The model under review builds one solid part; all positions refer to its coordinate system, in mm. A direction names the side the tool comes from. Coordinates: 2 decimals unless noted, no trailing zeros. Order: outer loops, then holes, each group sorted by start corner. A loop starts at its lowest first (then second) coordinate and runs counter-clockwise, first axis right, second up. Notation, with made-up numbers: (-33, 52) -> (-26, 52) arc R24 cw to (-26, 91) -> close; hole circle Ø3 at (81.5, 43). An arc over 180 degrees is marked (long way). Use one line per item in the form item = value. Start each with the question number.
(1) Mouldability with a two-part tool opening along Y and no side actions: class faces 1 (the flat face through (74, 58, -64)), 2 (the flat face through (74, 36, -64)), 3 (the flat face through (64, 32, -83)), 4 (the cylindrical face through (-84, 18, -15)) as +Y half, -Y half, draft (parallel to the pull), parting line (faces both ways), or undercut.
(2) Take a section at B-B (z = -129.5). State the section outline as (x, y) points.
(3) Insertion check: pin 1 Ø13 at (x, z) = (-77.5, -72) entering from +Y; pin 2 Ø2 at (y, z) = (35.5, -105) entering from -X; pin 3 Ø7 at (x, z) = (80, -15) entering from -Y; pin 4 Ø1 at (y, z) = (48.5, -93) entering from -X. Each pin has a flat end and moves straight along its axis. Give the tip position at first contact, or say it passes through.
(4) Take a section at A-A (x = -80). State the section outline as (y, z) points.
(5) Take a section at D-D (x = 0). State the section outline as (y, z) points.
(6) Take a section at C-C (y = 54). State the section outline as (x, z) points, then the cut area to 3 significant figures.
(7) Wall thickness on line 1 along Y through (x, z) = (64.5, -159.5); line 2 along X through (y, z) = (59.5, -161); line 3 along Z through (x, y) = (21, 47.5): over which ranges is each line inside the solid? List them lowest first.
(8) For faces 5 (the flat face through (64, 3, -83)), 6 (the flat face through (90, 47, -35)), 7 (the flat face through (-74, 7, -64)), list the 3-axis set-ups (+Z, -Z, +X, -X, +Y, -Y) from which the entire face can be reached by the end or side of a thin tool; tool diameter is ignored.
```python
from build123d import *

# Parameters (mm, degrees)
BOSS_EXTRUDE1_DEPTH = 65
SKETCH2_R           = 35
CUT_EXTRUDE1_DEPTH  = 65
SKETCH3_W           = 26
SKETCH3_H           = 7
CUT_EXTRUDE2_DEPTH  = 212.482859826
SKETCH4_R           = 4
CUT_EXTRUDE3_DEPTH  = 210.437341465
SKETCH5_W           = 26
SKETCH5_H           = 7
CUT_EXTRUDE4_DEPTH  = 212.482859826


with BuildPart() as part:
    # Sketch1 → Boss-Extrude1 (new body)
    with BuildSketch(Plane(origin=(0, 0, 0), x_dir=(1, 0, 0), z_dir=(0, 1, 0))):
        with BuildLine():
            Line((-90, 0), (90, 0))
            Line((90, 0), (90, 70))
            Line((90, 70), (69.444464042, 156.905307326))
            ThreePointArc((69.444464042, 156.905307326), (58.862371963, 173.528272565), (40.25, 180))
            Line((40.25, 180), (-40.25, 180))
            ThreePointArc((-40.25, 180), (-58.862371963, 173.528272565), (-69.444464042, 156.905307326))
            Line((-69.444464042, 156.905307326), (-90, 70))
            Line((-90, 70), (-90, 0))
        make_face()
    extrude(amount=BOSS_EXTRUDE1_DEPTH)

    # Sketch2 → Cut-Extrude1 (cut)
    with BuildSketch(Plane(origin=(0, 65, 0), x_dir=(1, 0, 0), z_dir=(0, 1, 0))):
        with Locations(Location((0, 117, 0), (0, 0, 270))):
            Circle(SKETCH2_R)
    extrude(amount=-CUT_EXTRUDE1_DEPTH, mode=Mode.SUBTRACT)

    # Sketch3 → Cut-Extrude2 (cut, through all)
    with BuildSketch(Plane.XY):
        with Locations((77, 3.5)):
            Rectangle(SKETCH3_W, SKETCH3_H)
        with Locations((77, 61.5)):
            Rectangle(SKETCH3_W, SKETCH3_H)
        with Locations((-77, 61.5)):
            Rectangle(SKETCH3_W, SKETCH3_H)
        with Locations((-77, 3.5)):
            Rectangle(SKETCH3_W, SKETCH3_H)
    extrude(amount=-CUT_EXTRUDE2_DEPTH, mode=Mode.SUBTRACT)

    # Sketch4 → Cut-Extrude3 (cut, through all)
    with BuildSketch(Plane.XZ.offset(-7)):
        with Locations((80, -15)):
            Circle(SKETCH4_R)
        with Locations((-80, -15)):
            Circle(SKETCH4_R)
    extrude(amount=-CUT_EXTRUDE3_DEPTH, mode=Mode.SUBTRACT)

    # Sketch5 → Cut-Extrude4 (cut, through all)
    with BuildSketch(Plane.XY):
        with Locations((-77, 32.5)):
            Rectangle(SKETCH5_W, SKETCH5_H)
        with Locations((77, 32.5)):
            Rectangle(SKETCH5_W, SKETCH5_H)
    extrude(amount=-CUT_EXTRUDE4_DEPTH, mode=Mode.SUBTRACT)


solid = part.part
```
Findings:
q1.face_1 = +Y half
q1.face_2 = undercut
q1.face_3 = undercut
q1.face_4 = draft
q2.outline = (-75.93, 7) -> (-64, 7) -> (-64, 0) -> (-32.69, 0) -> (-32.69, 65) -> (-64, 65) -> (-64, 58) -> (-75.93, 58) -> (-75.93, 36) -> (-64, 36) -> (-64, 29) -> (-75.93, 29) -> close; (32.69, 0) -> (64, 0) -> (64, 7) -> (75.93, 7) -> (75.93, 29) -> (64, 29) -> (64, 36) -> (75.93, 36) -> (75.93, 58) -> (64, 58) -> (64, 65) -> (32.69, 65) -> close
q3.pin_1 = 58
q3.pin_2 = -81.93
q3.pin_3 = through
q3.pin_4 = -84.68
q4.outline = (7, -112.28) -> (29, -112.28) -> (29, -19) -> (7, -19) -> close; (7, -11) -> (29, -11) -> (29, 0) -> (7, 0) -> close; (36, -112.28) -> (58, -112.28) -> (58, -19) -> (36, -19) -> close; (36, -11) -> (58, -11) -> (58, 0) -> (36, 0) -> close
q5.outline = (0, -180) -> (65, -180) -> (65, -152) -> (0, -152) -> close; (0, -82) -> (65, -82) -> (65, 0) -> (0, 0) -> close
q6.outline = (-90, -70) -> (-69.44, -156.91) arc R30 ccw to (-40.25, -180) -> (40.25, -180) arc R30 ccw to (69.44, -156.91) -> (90, -70) -> (90, 0) -> (-90, 0) -> close; hole circle Ø8 at (-80, -15); hole circle Ø70 at (0, -117); hole circle Ø8 at (80, -15)
q6.area = 25,400 mm²
q7.line_1 = 7 to 29, 36 to 58
q7.line_2 = -64 to 64
q7.line_3 = -180 to -145, -89 to 0
q8.face_5 = +Z, -Z, +X, -Y
q8.face_6 = +Z, -Z, +X, +Y, -Y
q8.face_7 = +Z, -Z, -X, -Y
